from build123d import *

# Parameters (mm, degrees)
EXTRUDE_1_DEPTH     = 280
SKETCH_2_R          = 10
CUT_EXTRUDE_1_DEPTH = 10


with BuildPart() as part:
    # 草图1 → 拉伸1 (new body)
    with BuildSketch(Plane.XY):
        with BuildLine():
            Line((0, 0), (0, 40))
            Line((0, 40), (3.99, 40))
            ThreePointArc((3.99, 40), (3.997071068, 39.997071068), (4, 39.99))
            Line((4, 39.99), (4, 9))
            ThreePointArc((4, 9), (5.464466094, 5.464466094), (9, 4))
            Line((9, 4), (39.99, 4))
            ThreePointArc((39.99, 4), (39.997071068, 3.997071068), (40, 3.99))
            Line((40, 3.99), (40, 0))
            Line((40, 0), (0, 0))
        make_face()
    extrude(amount=EXTRUDE_1_DEPTH)

    # 草图2 → 切除-拉伸1 (cut)
    with BuildSketch(Plane(origin=(0, 4, 0), x_dir=(1, 0, 0), z_dir=(0, 1, 0))):
        with Locations((45, -210)):
            Circle(SKETCH_2_R)
        with Locations((45, -70)):
            Circle(SKETCH_2_R)
    extrude(amount=-CUT_EXTRUDE_1_DEPTH, mode=Mode.SUBTRACT)


solid = part.part
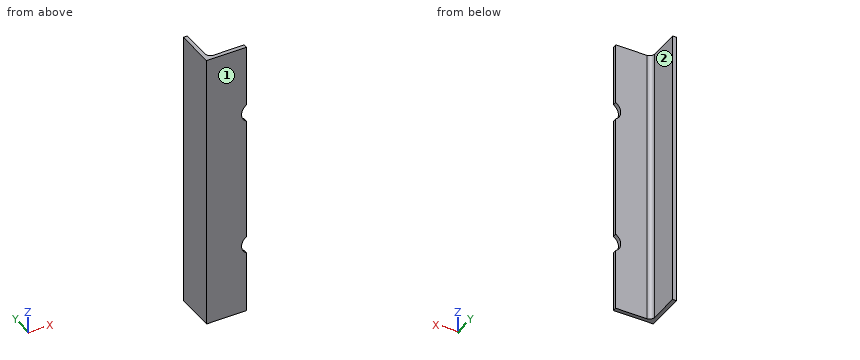
Can you work these out from the model? Positions are in its coordinate system, mm. Face numbers are marked on the shaded views. A direction names the side the tool comes from. Give positions to 0.01 mm unless a question says otherwise; leave off trailing zeros. Loops run counter-clockwise (first coordinate to the right, second up) from the corner with the lowest first, then second, coordinate; pieces in that order, holes last. Notation, with made-up numbers: (19.5, 78) - (49.5, 78) arc R32 ccw to (49.5, 112) - close; hole circle Ø2 at (-19, 61). An arc over 180 degrees is marked (long way). One line per item, written item: value.
(1) If we section it at B-B, the plane x = 24.5: List the corners of the cut face in (y, z) for me, plus the area to 3 significant figures.
Verdict:
outline: (0, 0) - (4, 0) - (4, 280) - (0, 280) - close
area: 1,120 mm^2
(2) I'm going to push flat-ended pins straight in: pin 1 (12 mm diameter, centred on y = 12, z = 120.5, fed in from +X); pin 2 (1.5 mm diameter, centred on y = 10.5, z = 43.5, fed in from +X); pin 3 (9.5 mm diameter, centred on x = 24, z = 166, fed in from +Y). Where does each tip first touch, or does it pass through?
Verdict:
pin 1: x = 5
pin 2: x = 4
pin 3: y = 4
(3) On a 3-axis mill with a long thin cutter (end or side, diameter ignored), from which of +Z, -Z, +X, -X, +Y, -Y can I reach the whole of each face in a straight line? I mean the marked faces 1 and 2. Say none if no direction works.
Verdict:
face 1: +Z, -Z, +X, -X, -Y
face 2: +Z, -Z, +X, +Y
(4) I need wall thicknesses on line 1 along Y through (x, z) = (17.5, 167.5); line 2 along X through (y, z) = (6, 20). Which ranges of each line are inside material? Lowest first, please.
Verdict:
line 1: 0 to 4
line 2: 0 to 5
